from build123d import *

# Parameters (mm, degrees)
SKETCH1_R           = 60
SKETCH1_R_2         = 55
BOSS_EXTRUDE1_DEPTH = 42
CHAMFER1_SIZE       = 2
CHAMFER2_SIZE       = 1


with BuildPart() as part:
    # Sketch1 → Boss-Extrude1 (new, symmetric)
    with BuildSketch(Plane.XY):
        with Locations(Location((0, 0, 0), (0, 0, 180))):
            Circle(SKETCH1_R)
        with Locations(Location((0, 0, 0), (0, 0, 180))):
            Circle(SKETCH1_R_2, mode=Mode.SUBTRACT)
    extrude(amount=BOSS_EXTRUDE1_DEPTH, both=True)

    # Chamfer1
    chamfer1_edges = [part.edges().sort_by_distance(p)[0] for p in [
        (60, 0, -42),
        (60, 0, 42),
    ]]
    chamfer(chamfer1_edges, length=CHAMFER1_SIZE)

    # Chamfer2
    chamfer2_edges = [part.edges().sort_by_distance(p)[0] for p in [
        (55, 0, -42),
        (55, 0, 42),
    ]]
    chamfer(chamfer2_edges, length=CHAMFER2_SIZE)


solid = part.part
Source: CAD feature listing. Evaluate the final solid. Frame: model axes, mm. Coordinates: 2 decimals unless noted, no trailing zeros. Loops run counter-clockwise (first coordinate to the right, second up) from the corner with the lowest first, then second, coordinate; pieces in that order, holes last. Notation, with made-up numbers: (52.5, 55.5) -> (103.5, 55.5) arc R17 cw to (103.5, 59.5) -> close; hole circle Ø7 at (57, 50). An arc over 180 degrees is marked (long way). Answer in a Markdown table with one row per item. Add a question column.
Q1. Contact query for flat-ended pins moving along their axis: pin 1 Ø8 at (y, z) = (27.5, -8) entering from -X; pin 2 Ø5 at (y, z) = (-43, 21.5) entering from -X; pin 3 Ø8 at (x, y) = (9, 48) entering from +Z; pin 4 Ø12 at (x, z) = (-28, -9.5) entering from +Y. Output: stop coordinate, or through.
Q2. Ray query, line 1 along Y through (x, z) = (0, -16.5); line 2 along Y through (x, z) = (-15.5, -35); line 3 along X through (y, z) = (3.5, 14.5). Return the intervals inside material, ascending.
Q3. Pull-direction query (Y, two-part tool) for faces 1 (the face through (-25.379, 48.794, -0.574)), 2 (the face through (-32.26, -50.59, 0.56)), 3 (the face through (48, -30, 42)); classes: pulls with the +Y half, pulls with the -Y half, needs draft (parallel to the pull), parting line crosses it, or undercut.
Q4. Section C-C on z = 35. Return the cut outline in (x, y).
Q5. Section A-A on y = 0. Return the cut outline in (x, z), and give its area (3 significant figures).
Computed values:
| question | item | result |
|---|---|---|
| 1 | pin 1 | stops at x = -55.21 |
| 1 | pin 2 | stops at x = -44.27 |
| 1 | pin 3 | passes through |
| 1 | pin 4 | stops at y = 55.82 |
| 2 | line 1 | y = -60 to -55, 55 to 60 |
| 2 | line 2 | y = -57.96 to -52.77, 52.77 to 57.96 |
| 2 | line 3 | x = -59.9 to -54.89, 54.89 to 59.9 |
| 3 | face 1 | undercut |
| 3 | face 2 | parting line crosses it |
| 3 | face 3 | needs draft |
| 4 | outline | circle Ø120 at (0, 0); hole circle Ø110 at (0, 0) |
| 5 | outline | (-60, -40) -> (-58, -42) -> (-56, -42) -> (-55, -41) -> (-55, 41) -> (-56, 42) -> (-58, 42) -> (-60, 40) -> close; (55, -41) -> (56, -42) -> (58, -42) -> (60, -40) -> (60, 40) -> (58, 42) -> (56, 42) -> (55, 41) -> close |
| 5 | area | 830 mm^2 |
